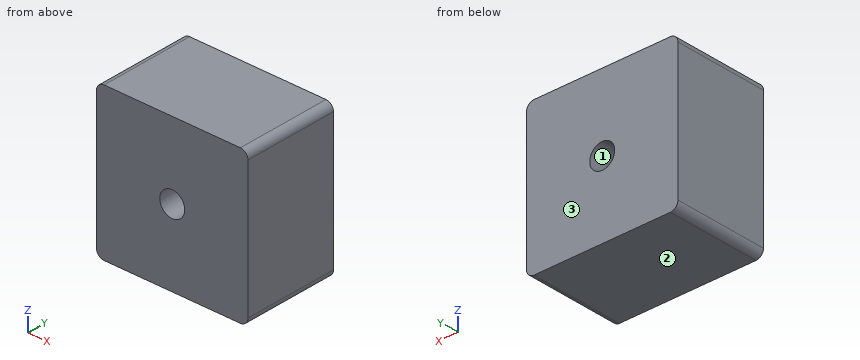
from build123d import *

# Parameters (mm, degrees)
SKETCH1_W           = 20
SKETCH1_H           = 20
BOSS_EXTRUDE1_DEPTH = 12.5
M4_TAPPED_HOLE1_D   = 3.3
FILLET1_R           = 1


with BuildPart() as part:
    # Sketch1 → Boss-Extrude1 (new body)
    with BuildSketch(Plane(origin=(0, 0, 0), x_dir=(1, 0, 0), z_dir=(0, 1, 0))):
        Rectangle(SKETCH1_W, SKETCH1_H)
    extrude(amount=BOSS_EXTRUDE1_DEPTH)

    # M4 Tapped Hole1 (through all)
    with Locations(Plane(origin=(0, 12.5, 0), x_dir=(1, 0, 0), z_dir=(0, 1, 0))):
        with Locations((0, 0)):
            Hole(M4_TAPPED_HOLE1_D / 2)

    # Fillet1
    fillet1_edges = [part.edges().sort_by_distance(p)[0] for p in [
        (10, 6.25, 10),
        (-10, 6.25, 10),
        (-10, 6.25, -10),
        (10, 6.25, -10),
    ]]
    fillet(fillet1_edges, radius=FILLET1_R)


solid = part.part
Design review of the part built by this model. Coordinates are the model's own, in mm. Face numbers are marked on the shaded views. Give positions to 0.01 mm unless a question says otherwise; leave off trailing zeros. Loops run counter-clockwise (first coordinate to the right, second up) from the corner with the lowest first, then second, coordinate; pieces in that order, holes last. Notation, with made-up numbers: (-35, -5) - (-21, -5) arc R8 ccw to (-21, -1) - close; hole circle Ø5 at (78, -35.5). An arc over 180 degrees is marked (long way). Write item = value, one per line.
1) Draft analysis for pull direction Z (two halves, no side actions). For the marked faces 1, 2 and 3, state which applies: +Z half, -Z half, draft (parallel to the pull), parting line (faces both ways), or undercut.
Result sheet:
face_1 = undercut
face_2 = -Z half
face_3 = draft
2) Clearance check with a flat-ended pin moving along its axis: pin 1 Ø2 at (x, z) = (0, 0) entering from +Y. State where the tip first meets the part, or that it passes through.
Result sheet:
pin_1 = through
3) To check wall thickness, follow line 1 (Z direction, x = 0, y = 10); line 2 (X direction, y = 11.5, z = 0.75); line 3 (X direction, y = 3.25, z = -0.25). State the ranges of each line that lie inside material, in increasing order.
Result sheet:
line_1 = -10 to -1.65, 1.65 to 10
line_2 = -10 to -1.47, 1.47 to 10
line_3 = -10 to -1.63, 1.63 to 10
4) Take a section at A-A on z = 0. State the section outline as (x, y) points, and give its area (3 significant figures).
Result sheet:
outline = (-10, 0) - (-1.65, 0) - (-1.65, 12.5) - (-10, 12.5) - close; (1.65, 0) - (10, 0) - (10, 12.5) - (1.65, 12.5) - close
area = 209 mm2
5) Take a section at C-C on y = 3.25. State the section outline as (x, z) points, and give its area (3 significant figures).
Result sheet:
outline = (-10, -9) arc R1 ccw to (-9, -10) - (9, -10) arc R1 ccw to (10, -9) - (10, 9) arc R1 ccw to (9, 10) - (-9, 10) arc R1 ccw to (-10, 9) - close; hole circle Ø3.3 at (0, 0)
area = 391 mm2
6) Take a section at B-B on x = 0. State the section outline as (y, z) points, and give its area (3 significant figures).
Result sheet:
outline = (0, -10) - (12.5, -10) - (12.5, -1.65) - (0, -1.65) - close; (0, 1.65) - (12.5, 1.65) - (12.5, 10) - (0, 10) - close
area = 209 mm2
